CAD build for the part. Positions are in the model's coordinates, mm. Round coordinates to 2 decimals unless told otherwise and drop trailing zeros. Order: outer loops, then holes, each group sorted by start corner. A loop starts at its lowest first (then second) coordinate and runs counter-clockwise, first axis right, second up. Notation, with made-up numbers: (-25.5, -20) - (11.5, -20) arc R15 ccw to (11.5, -16) - close; hole circle Ø7 at (-26.5, 42.5). An arc over 180 degrees is marked (long way). Write item = value, one per line.
from build123d import *

# Parameters (mm, degrees)
SKETCH1_W              = 130
SKETCH1_H              = 50
BOSS_EXTRUDE1_DEPTH    = 15
M12_TAPPED_HOLE1_D     = 10.2
M12_TAPPED_HOLE1_DEPTH = 29.25
M12_TAPPED_HOLE1_TIP   = 3.064389157


with BuildPart() as part:
    # Sketch1 → Boss-Extrude1 (new body)
    with BuildSketch(Plane.XY):
        Rectangle(SKETCH1_W, SKETCH1_H)
    extrude(amount=BOSS_EXTRUDE1_DEPTH)

    # M12 Tapped Hole1
    with Locations(Plane.XY.offset(15)):
        with Locations((-30, -10), (30, -10)):
            Hole(M12_TAPPED_HOLE1_D / 2, depth=M12_TAPPED_HOLE1_DEPTH)
            with Locations((0, 0, -(M12_TAPPED_HOLE1_DEPTH + M12_TAPPED_HOLE1_TIP / 2))):  # 118° drill point
                Cone(0, M12_TAPPED_HOLE1_D / 2, M12_TAPPED_HOLE1_TIP, mode=Mode.SUBTRACT)


solid = part.part
(1) Band-saw the part on B-B on y = -10. List the corners of the cut face in (x, z).
Solved:
outline = (-65, 0) - (-35.1, 0) - (-35.1, 15) - (-65, 15) - close; (-24.9, 0) - (24.9, 0) - (24.9, 15) - (-24.9, 15) - close; (35.1, 0) - (65, 0) - (65, 15) - (35.1, 15) - close
(2) Band-saw the part on D-D on x = -32. List the corners of the cut face in (y, z), plus the area to 3 significant figures.
Solved:
outline = (-25, 0) - (-14.69, 0) - (-14.69, 15) - (-25, 15) - close; (-5.31, 0) - (25, 0) - (25, 15) - (-5.31, 15) - close
area = 609 mm²
(3) Band-saw the part on C-C on z = 4.25. List the corners of the cut face in (x, y), plus the area to 3 significant figures.
Solved:
outline = (-65, -25) - (65, -25) - (65, 25) - (-65, 25) - close; hole circle Ø10.2 at (-30, -10); hole circle Ø10.2 at (30, -10)
area = 6,340 mm²
(4) Band-saw the part on A-A on x = 30. List the corners of the cut face in (y, z).
Solved:
outline = (-25, 0) - (-15.1, 0) - (-15.1, 15) - (-25, 15) - close; (-4.9, 0) - (25, 0) - (25, 15) - (-4.9, 15) - close
(5) Probe line 1 along Y through (x, z) = (-30, 10.5); line 2 along X through (y, z) = (-14, 2.5); line 3 along X through (y, z) = (-13, 14). List the from-to ranges inside material, lowest first.
Solved:
line_1 = -25 to -15.1, -4.9 to 25
line_2 = -65 to -33.16, -26.84 to 26.84, 33.16 to 65
line_3 = -65 to -34.12, -25.88 to 25.88, 34.12 to 65
